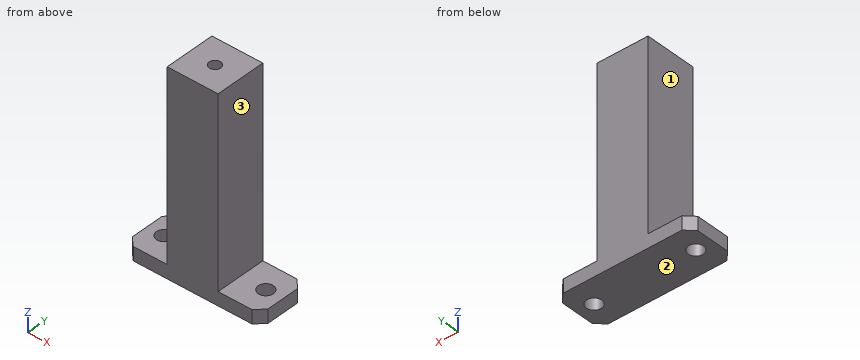
from build123d import *

# Parameters (mm, degrees)
SKETCH1_R             = 4.5
BOSS_EXTRUDE1_DEPTH   = 8
SKETCH2_W             = 30
SKETCH2_H             = 30
BOSS_EXTRUDE2_DEPTH   = 110
SKETCH3_R             = 1.5
CUT_EXTRUDE1_DEPTH    = 10
M8_TAPPED_HOLE1_D     = 6.8
M8_TAPPED_HOLE1_DEPTH = 25
M8_TAPPED_HOLE1_TIP   = 2.042926105


with BuildPart() as part:
    # Sketch1 → Boss-Extrude1 (new body)
    with BuildSketch(Plane.XY):
        Polygon((-40, 10), (-35, 15), (35, 15), (40, 10), (40, -10), (35, -15), (-35, -15), (-40, -10), align=None)
        with Locations((-30, 0)):
            Circle(SKETCH1_R, mode=Mode.SUBTRACT)
        with Locations((30, 0)):
            Circle(SKETCH1_R, mode=Mode.SUBTRACT)
    extrude(amount=BOSS_EXTRUDE1_DEPTH)

    # Sketch2 → Boss-Extrude2 (add)
    with BuildSketch(Plane.XY.offset(8)):
        Rectangle(SKETCH2_W, SKETCH2_H)
    extrude(amount=BOSS_EXTRUDE2_DEPTH)

    # Sketch3 → Cut-Extrude1 (cut)
    with BuildSketch(Plane.XY.offset(118)):
        Circle(SKETCH3_R)
    extrude(amount=-CUT_EXTRUDE1_DEPTH, mode=Mode.SUBTRACT)

    # M8 Tapped Hole1
    with Locations(Plane.XY.offset(118)):
        with Locations((0, 0)):
            Hole(M8_TAPPED_HOLE1_D / 2, depth=M8_TAPPED_HOLE1_DEPTH)
            with Locations((0, 0, -(M8_TAPPED_HOLE1_DEPTH + M8_TAPPED_HOLE1_TIP / 2))):  # 118° drill point
                Cone(0, M8_TAPPED_HOLE1_D / 2, M8_TAPPED_HOLE1_TIP, mode=Mode.SUBTRACT)


solid = part.part
Input: part model. Units: mm. Frame: model coordinates. Face numbers are marked on the shaded views. A direction names the side the tool comes from. Give positions to 0.01 mm unless a question says otherwise; leave off trailing zeros. Order: outer loops, then holes, each group sorted by start corner. A loop starts at its lowest first (then second) coordinate and runs counter-clockwise, first axis right, second up. Notation, with made-up numbers: M 3,62.25 L 49,62.25 A30 ccw 49,90.25 Z; hole C -5.5,55.5 d6. An arc over 180 degrees is marked long. Answer as a JSON object with one key per item and string values.
1. Reachability of the marked faces 1, 2 and 3 from +Z, -Z, +X, -X, +Y, -Y: full face, straight path, thin tool, end or side. Return the list, or none.
Result sheet:
{"face 1": "+Z, -X, +Y, -Y", "face 2": "-Z, +X, -X, +Y, -Y", "face 3": "+Z, +X, +Y, -Y"}
2. Cut plane C-C, the plane z = 19. Output: boundary loops of the cut face in (x, y).
Result sheet:
{"outline": "M -15,-15 L 15,-15 L 15,15 L -15,15 Z"}
3. First-contact query: P1, Ø7.5, axis at x = 31.5, y = -1, coming from the +Z side; P2, Ø6, axis at y = 9.5, z = 63, coming from the -X side; P3, Ø3, axis at y = 0.5, z = 87, coming from the +X side. Flat tips, straight axial feed; report the tip coordinate or a pass-through.
Result sheet:
{"P1": "z = 8", "P2": "x = -15", "P3": "x = 15"}
4. Cut plane A-A, the plane x = 30. Output: boundary loops of the cut face in (y, z).
Result sheet:
{"outline": "M -15,0 L -4.5,0 L -4.5,8 L -15,8 Z; M 4.5,0 L 15,0 L 15,8 L 4.5,8 Z"}
5. Cut plane B-B, the plane z = 101.5. Output: boundary loops of the cut face in (x, y).
Result sheet:
{"outline": "M -15,-15 L 15,-15 L 15,15 L -15,15 Z; hole C 0,0 d6.8"}
6. Ray query, line 1 (Y direction, x = 30, z = 4.5); line 2 (Z direction, x = -24, y = 12.25); line 3 (X direction, y = -9.75, z = 46). Return the intervals inside material, ascending. Write a range as [from, to].
Result sheet:
{"line 1": "[-15, -4.5], [4.5, 15]", "line 2": "[0, 8]", "line 3": "[-15, 15]"}
